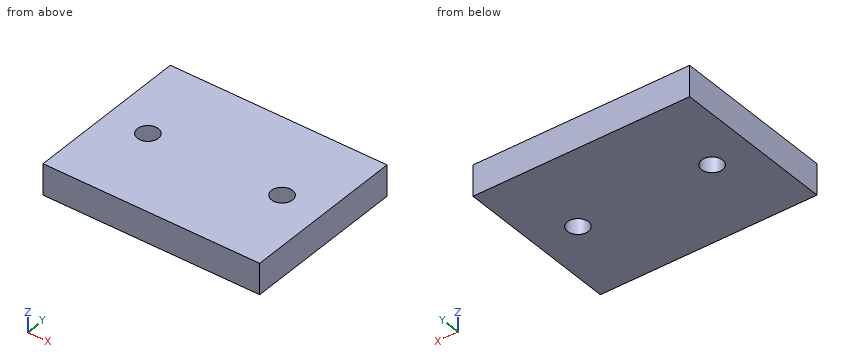
```python
from build123d import *

# Parameters (mm, degrees)
SKETCH_1_W              = 105
SKETCH_1_H              = 80
EXTRUDE_1_DEPTH         = 15
HOLE_WIZARD_M12_1_D     = 10.2
HOLE_WIZARD_M12_1_DEPTH = 29.25
HOLE_WIZARD_M12_1_TIP   = 3.064389157


with BuildPart() as part:
    # 草图1 → 凸台-拉伸1 (new body)
    with BuildSketch(Plane.XY):
        Rectangle(SKETCH_1_W, SKETCH_1_H)
    extrude(amount=EXTRUDE_1_DEPTH)

    # M12 螺纹孔1
    with Locations(Plane.XY.offset(15)):
        with Locations((-32.5, 0), (32.5, 0)):
            Hole(HOLE_WIZARD_M12_1_D / 2, depth=HOLE_WIZARD_M12_1_DEPTH)
            with Locations((0, 0, -(HOLE_WIZARD_M12_1_DEPTH + HOLE_WIZARD_M12_1_TIP / 2))):  # 118° drill point
                Cone(0, HOLE_WIZARD_M12_1_D / 2, HOLE_WIZARD_M12_1_TIP, mode=Mode.SUBTRACT)


solid = part.part
```
Build history of the part. All positions in model axes, mm. Round coordinates to 2 decimals unless told otherwise and drop trailing zeros. Write each loop counter-clockwise with the first axis right and the second up, starting at its lowest first coordinate (ties: lowest second). Pieces come first, ordered by that corner, then holes.
1) Band-saw the part on A-A, the plane x = -32.5. List the corners of the cut face in (y, z), and give its area (3 significant figures).
2) Band-saw the part on D-D, the plane x = 36.5. List the corners of the cut face in (y, z), and give its area (3 significant figures).
3) Band-saw the part on C-C, the plane z = 5.5. List the corners of the cut face in (x, y), and give its area (3 significant figures).
4) Drill centre line: probe 1 along Y at (x, z) = (-32.5, 11.5). Where is it in solid material? Low to high.
5) Band-saw the part on B-B, the plane y = 0. List the corners of the cut face in (x, z), and give its area (3 significant figures).
Ans:
1. outline: (-40, 0) - (-5.1, 0) - (-5.1, 15) - (-40, 15) - close; (5.1, 0) - (40, 0) - (40, 15) - (5.1, 15) - close
1. area: 1,050 mm2
2. outline: (-40, 0) - (-3.16, 0) - (-3.16, 15) - (-40, 15) - close; (3.16, 0) - (40, 0) - (40, 15) - (3.16, 15) - close
2. area: 1,110 mm2
3. outline: (-52.5, -40) - (52.5, -40) - (52.5, 40) - (-52.5, 40) - close; hole circle Ø10.2 at (-32.5, 0); hole circle Ø10.2 at (32.5, 0)
3. area: 8,240 mm2
4. probe 1: y = -40 to -5.1, 5.1 to 40
5. outline: (-52.5, 0) - (-37.6, 0) - (-37.6, 15) - (-52.5, 15) - close; (-27.4, 0) - (27.4, 0) - (27.4, 15) - (-27.4, 15) - close; (37.6, 0) - (52.5, 0) - (52.5, 15) - (37.6, 15) - close
5. area: 1,270 mm2
